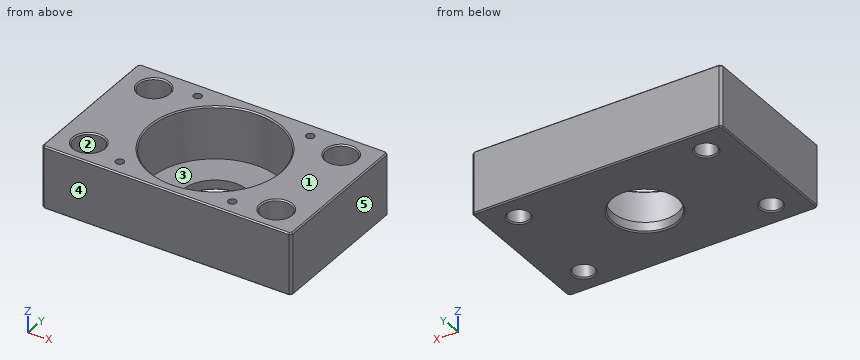
from build123d import *

# Parameters (mm, degrees)
SKETCH_1_W          = 100
SKETCH_1_H          = 60
EXTRUDE_1_DEPTH     = 25
SKETCH_2_R          = 13
CUT_EXTRUDE_1_DEPTH = 64.442887702
SKETCH_3_R          = 6
CUT_EXTRUDE_2_DEPTH = 12
SKETCH_4_R          = 4.1
CUT_EXTRUDE_3_DEPTH = 64.442887702
CHAMFER_1_SIZE      = 1
CHAMFER_4_SIZE      = 0.5
SKETCH_8_R          = 26
CUT_EXTRUDE_5_DEPTH = 21
CHAMFER_5_SIZE      = 0.5
SKETCH_9_R          = 1.65
CUT_EXTRUDE_6_DEPTH = 15


with BuildPart() as part:
    # 草图1 → 凸台-拉伸1 (new body)
    with BuildSketch(Plane.XY):
        Rectangle(SKETCH_1_W, SKETCH_1_H)
    extrude(amount=EXTRUDE_1_DEPTH)

    # 草图2 → 切除-拉伸1 (cut, through all)
    with BuildSketch(Plane.XY.offset(25)):
        Circle(SKETCH_2_R)
    extrude(amount=-CUT_EXTRUDE_1_DEPTH, mode=Mode.SUBTRACT)

    # 草图3 → 切除-拉伸2 (cut)
    with BuildSketch(Plane.XY.offset(25)):
        with Locations((-37.5, 20)):
            Circle(SKETCH_3_R)
        with Locations((-37.5, -20)):
            Circle(SKETCH_3_R)
        with Locations((37.5, -20)):
            Circle(SKETCH_3_R)
        with Locations((37.5, 20)):
            Circle(SKETCH_3_R)
    extrude(amount=-CUT_EXTRUDE_2_DEPTH, mode=Mode.SUBTRACT)

    # 草图4 → 切除-拉伸3 (cut, through all)
    with BuildSketch(Plane.XY.offset(25)):
        with Locations((-37.5, 20)):
            Circle(SKETCH_4_R)
        with Locations((-37.5, -20)):
            Circle(SKETCH_4_R)
        with Locations((37.5, 20)):
            Circle(SKETCH_4_R)
        with Locations((37.5, -20)):
            Circle(SKETCH_4_R)
    extrude(amount=-CUT_EXTRUDE_3_DEPTH, mode=Mode.SUBTRACT)

    # 倒角1
    chamfer_1_edges = [part.edges().sort_by_distance(p)[0] for p in [
        (50, -30, 12.5),
        (-50, -30, 12.5),
        (-50, 30, 12.5),
        (50, 30, 12.5),
    ]]
    chamfer(chamfer_1_edges, length=CHAMFER_1_SIZE)

    # 倒角4
    chamfer_4_edges = [part.edges().sort_by_distance(p)[0] for p in [
        (-13, 0, 0),
        (-41.6, -20, 0),
        (33.4, 20, 0),
        (33.4, -20, 0),
        (-41.6, 20, 0),
        (-50, 0, 0),
        (50, 0, 0),
        (0, -30, 0),
        (0, 30, 0),
        (-49.5, -29.5, 0),
        (49.5, -29.5, 0),
        (49.5, 29.5, 0),
        (-49.5, 29.5, 0),
    ]]
    chamfer(chamfer_4_edges, length=CHAMFER_4_SIZE)

    # 草图8 → 切除-拉伸5 (cut)
    with BuildSketch(Plane.XY.offset(25)):
        Circle(SKETCH_8_R)
    extrude(amount=-CUT_EXTRUDE_5_DEPTH, mode=Mode.SUBTRACT)

    # 倒角5
    chamfer_5_edges = [part.edges().sort_by_distance(p)[0] for p in [
        (-26, 0, 25),
        (31.5, 20, 25),
        (31.5, -20, 25),
        (-43.5, -20, 25),
        (-43.5, 20, 25),
        (-50, 0, 25),
        (0, 30, 25),
        (50, 0, 25),
        (0, -30, 25),
        (-49.5, -29.5, 25),
        (49.5, -29.5, 25),
        (49.5, 29.5, 25),
        (-49.5, 29.5, 25),
    ]]
    chamfer(chamfer_5_edges, length=CHAMFER_5_SIZE)

    # 草图9 → 切除-拉伸6 (cut)
    with BuildSketch(Plane.XY.offset(25)):
        with Locations((22.5, -24)):
            Circle(SKETCH_9_R)
        with Locations((22.5, 24)):
            Circle(SKETCH_9_R)
        with Locations((-22.5, 24)):
            Circle(SKETCH_9_R)
        with Locations((-22.5, -24)):
            Circle(SKETCH_9_R)
    extrude(amount=-CUT_EXTRUDE_6_DEPTH, mode=Mode.SUBTRACT)


solid = part.part
Read the model definition and answer for the solid it produces. Units are mm, in the model's axes. Face numbers are marked on the shaded views. A direction names the side the tool comes from. Coordinates: 2 decimals unless noted, no trailing zeros. Write each loop counter-clockwise with the first axis right and the second up, starting at its lowest first coordinate (ties: lowest second). Pieces come first, ordered by that corner, then holes. Notation, with made-up numbers: (37, -38.5) -> (90, -38.5) arc R21 cw to (90, -20.5) -> close; hole circle Ø9 at (25.5, -6). An arc over 180 degrees is marked (long way). Return JSON: item names as keys, results as strings.
(1) Each of these flat-tipped pins is pushed along its axis until it touches: P1, Ø9.5, axis at x = 37.5, y = 20, coming from the +Z side; P2, Ø1.5, axis at x = -33, y = -23.5, coming from the +Z side; P3, Ø1, axis at x = -6.5, y = 20.5, coming from the +Z side. Where does it stop, or does it pass through?
Answers below:
{"P1": "z = 13", "P2": "z = 24.95", "P3": "z = 4"}
(2) The part is cut by section A-A on x = 0. Give the vertices of the cut face in (y, z), then the cut area to 3 significant figures.
Answers below:
{"outline": "(-30, 0.5) -> (-29.5, 0) -> (-13.5, 0) -> (-13, 0.5) -> (-13, 4) -> (-26, 4) -> (-26, 24.5) -> (-26.5, 25) -> (-29.5, 25) -> (-30, 24.5) -> close; (13, 0.5) -> (13.5, 0) -> (29.5, 0) -> (30, 0.5) -> (30, 24.5) -> (29.5, 25) -> (26.5, 25) -> (26, 24.5) -> (26, 4) -> (13, 4) -> close", "area": "303 mm^2"}
(3) Consider line 1 along Y through (x, z) = (-22.5, 19.5); line 2 along Y through (x, z) = (37.5, 17.5); line 3 along Y through (x, z) = (-37.5, 9.5). Determine where each line is inside the solid, lowest interval first. Write a range as from..to.
Answers below:
{"line 1": "-30..-25.65, -22.35..-13.03, 13.03..22.35, 25.65..30", "line 2": "-30..-26, -14..14, 26..30", "line 3": "-30..-24.1, -15.9..15.9, 24.1..30"}
(4) The part is cut by section B-B on z = 2.25. Give the vertices of the cut face in (x, y), then the cut area to 3 significant figures.
Answers below:
{"outline": "(-50, -29) -> (-49, -30) -> (49, -30) -> (50, -29) -> (50, 29) -> (49, 30) -> (-49, 30) -> (-50, 29) -> close; hole circle Ø8.2 at (-37.5, -20); hole circle Ø8.2 at (-37.5, 20); hole circle Ø26 at (0, 0); hole circle Ø8.2 at (37.5, -20); hole circle Ø8.2 at (37.5, 20)", "area": "5,260 mm^2"}
(5) Which of the six approach directions +Z, -Z, +X, -X, +Y, -Y give full straight-line access (tool end or side, diameter ignored) to the marked faces 1 and 2?
Answers below:
{"face 1": "+Z, +X, -X, +Y, -Y", "face 2": "+Z"}
(6) The part is cut by section C-C on x = 37.5. State how many separate pieces and enclosed holes the cut face has, then the cut area to 3 significant figures.
Answers below:
{"separate pieces": "3", "enclosed holes": "0", "area": "997 mm^2"}
(7) For a pull along Y with two mould halves and no side action, classify the marked faces 3, 4 and 5 as pulls with the +Y half, pulls with the -Y half, needs draft (parallel to the pull), parting line crosses it, or undercut.
Answers below:
{"face 3": "undercut", "face 4": "pulls with the -Y half", "face 5": "needs draft"}
